Work out the finished part from the listing and answer in its coordinate system (mm). Face numbers are marked on the shaded views. A direction names the side the tool comes from. Coordinates: 2 decimals unless noted, no trailing zeros. Order: outer loops, then holes, each group sorted by start corner. A loop starts at its lowest first (then second) coordinate and runs counter-clockwise, first axis right, second up. Notation, with made-up numbers: (63.25, -7) -> (95.25, -7) arc R28 cw to (95.25, 22) -> close; hole circle Ø8 at (81, -21.75). An arc over 180 degrees is marked (long way). Use one line per item in the form item = value.
from build123d import *

# Parameters (mm, degrees)
SKETCH1_W           = 80
SKETCH1_H           = 50
BOSS_EXTRUDE1_DEPTH = 166
FILLET1_R           = 5
SHELL1_T            = -3


with BuildPart() as part:
    # Sketch1 → Boss-Extrude1 (new body)
    with BuildSketch(Plane.XY):
        Rectangle(SKETCH1_W, SKETCH1_H)
    extrude(amount=BOSS_EXTRUDE1_DEPTH)

    # Fillet1
    fillet1_edges = [part.edges().sort_by_distance(p)[0] for p in [
        (-40, 25, 83),
        (40, 25, 83),
        (40, -25, 83),
        (-40, -25, 83),
    ]]
    fillet(fillet1_edges, radius=FILLET1_R)

    # Shell1
    shell1_openings = [part.faces().sort_by_distance(p)[0] for p in [
        (0, 0, 166),
        (0, 0, 0),
    ]]
    offset(amount=SHELL1_T, openings=shell1_openings, kind=Kind.INTERSECTION)


solid = part.part
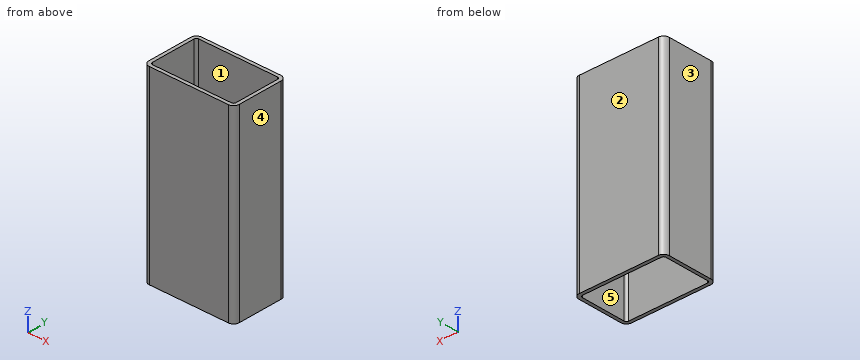
(1) Section A-A on y = 2 is taken. Write down the section's boundary in (x, z), plus the area to 3 significant figures.
Data:
outline = (-40, 0) -> (-37, 0) -> (-37, 166) -> (-40, 166) -> close; (37, 0) -> (40, 0) -> (40, 166) -> (37, 166) -> close
area = 996 mm²
(2) Section B-B on x = -26 is taken. Write down the section's boundary in (y, z).
Data:
outline = (-25, 0) -> (-22, 0) -> (-22, 166) -> (-25, 166) -> close; (22, 0) -> (25, 0) -> (25, 166) -> (22, 166) -> close
(3) Section C-C on z = 29 is taken. Write down the section's boundary in (x, y), plus the area to 3 significant figures.
Data:
outline = (-40, -20) arc R5 ccw to (-35, -25) -> (35, -25) arc R5 ccw to (40, -20) -> (40, 20) arc R5 ccw to (35, 25) -> (-35, 25) arc R5 ccw to (-40, 20) -> close; hole (-37, -20) arc R2 ccw to (-35, -22) -> (35, -22) arc R2 ccw to (37, -20) -> (37, 20) arc R2 ccw to (35, 22) -> (-35, 22) arc R2 ccw to (-37, 20) -> close
area = 726 mm²
(4) Which of the six approach directions +Z, -Z, +X, -X, +Y, -Y give full straight-line access (tool end or side, diameter ignored) to the marked faces 4 and 5?
Data:
face_4 = +Z, -Z, +X, +Y, -Y
face_5 = +Z, -Z
(5) The mould has two halves that part along X. Classify the marked faces 1, 2 and 3: released by +X, released by -X, zero draft, split by the parting line, or undercut.
Data:
face_1 = undercut
face_2 = zero draft
face_3 = released by -X
(6) Straight lines are drawn through the part: line 1 along Y through (x, z) = (-2, 43.5); line 2 along X through (y, z) = (-3, 151.5); line 3 along Y through (x, z) = (36, 134). For each, find the intervals that lie inside material, in ascending order.
Data:
line_1 = -25 to -22, 22 to 25
line_2 = -40 to -37, 37 to 40
line_3 = -24.9 to -21.73, 21.73 to 24.9
